```python
from build123d import *

# Parameters (mm, degrees)
BASE_BLOCK_DEPTH        = 26
UPPER_GUIDE_BLOCK_DEPTH = 30
GUIDE_SLOTS_SKETCH_W    = 26
GUIDE_SLOTS_SKETCH_H    = 5
GUIDE_SLOTS_SKETCH_W_2  = 15
GUIDE_SLOTS_SKETCH_H_2  = 20
GUIDE_SLOTS_CUT_DEPTH   = 30
OFFSET_BOSS_DEPTH       = 20
TOP_BORE_SKETCH_R       = 10
TOP_BORE_DEPTH          = 83
POCKET_SKETCH_W         = 15
POCKET_SKETCH_H         = 20
POCKET_8MM_DEEP_DEPTH   = 8
SIDE_ARCH_CUT_DEPTH     = 121
BEARING_ARCH_SKETCH_R   = 20
BEARING_ARCH_CUT_DEPTH  = 121


with BuildPart() as part:
    # Base Profile Sketch → Base Block (new body)
    with BuildSketch(Plane(origin=(0, 0, 0), x_dir=(1, 0, 0), z_dir=(0, 1, 0))):
        Polygon((50, 0), (50, 30), (-50, 30), (-50, -30), (50, -30), align=None)
    extrude(amount=BASE_BLOCK_DEPTH)

    # Upper Block Sketch → Upper Guide Block (add)
    with BuildSketch(Plane(origin=(0, 26, 0), x_dir=(1, 0, 0), z_dir=(0, 1, 0))):
        Polygon((35, 0), (35, 20), (-35, 20), (-35, -20), (35, -20), align=None)
    extrude(amount=UPPER_GUIDE_BLOCK_DEPTH)

    # Guide Slots Sketch → Guide Slots Cut (cut)
    with BuildSketch(Plane(origin=(0, 56, 0), x_dir=(1, 0, 0), z_dir=(0, 1, 0))):
        Polygon((35, 0), (35, 10), (20, 10), (20, -10), (35, -10), align=None)
        with Locations((0, -17.5)):
            Rectangle(GUIDE_SLOTS_SKETCH_W, GUIDE_SLOTS_SKETCH_H)
        with Locations((-27.5, 0)):
            Rectangle(GUIDE_SLOTS_SKETCH_W_2, GUIDE_SLOTS_SKETCH_H_2)
        with Locations((0, 17.5)):
            Rectangle(GUIDE_SLOTS_SKETCH_W, GUIDE_SLOTS_SKETCH_H)
    extrude(amount=-GUIDE_SLOTS_CUT_DEPTH, mode=Mode.SUBTRACT)

    # Offset Boss Sketch → Offset Boss (add)
    with BuildSketch(Plane.XY.offset(10)):
        Polygon((-20, 56), (-35, 26), (-20, 26), align=None)
        Polygon((20, 56), (35, 26), (20, 26), align=None)
    extrude(amount=-OFFSET_BOSS_DEPTH)

    # Top Bore Sketch → Top Bore (cut)
    with BuildSketch(Plane(origin=(0, 56, 0), x_dir=(1, 0, 0), z_dir=(0, 1, 0))):
        with Locations(Location((0, 0, 0), (0, 0, 270))):
            Circle(TOP_BORE_SKETCH_R)
    extrude(amount=-TOP_BORE_DEPTH, mode=Mode.SUBTRACT)

    # Pocket Sketch → Pocket 8mm Deep (cut)
    with BuildSketch(Plane(origin=(0, 26, 0), x_dir=(1, 0, 0), z_dir=(0, 1, 0))):
        with Locations((42.5, 0)):
            Rectangle(POCKET_SKETCH_W, POCKET_SKETCH_H)
        with Locations((-42.5, 0)):
            Rectangle(POCKET_SKETCH_W, POCKET_SKETCH_H)
    extrude(amount=-POCKET_8MM_DEEP_DEPTH, mode=Mode.SUBTRACT)

    # Side Arch Sketch → Side Arch Cut (cut)
    with BuildSketch(Plane.ZY.offset(50)):
        with BuildLine():
            Line((-15, 0), (15, 0))
            ThreePointArc((15, 0), (0, 15), (-15, 0))
        make_face()
    extrude(amount=-SIDE_ARCH_CUT_DEPTH, mode=Mode.SUBTRACT)

    # Bearing Arch Sketch → Bearing Arch Cut (cut)
    with BuildSketch(Plane(origin=(0, 0, -30), x_dir=(-1, 0, 0), z_dir=(0, 0, -1))):
        Circle(BEARING_ARCH_SKETCH_R)
    extrude(amount=-BEARING_ARCH_CUT_DEPTH, mode=Mode.SUBTRACT)


solid = part.part
```
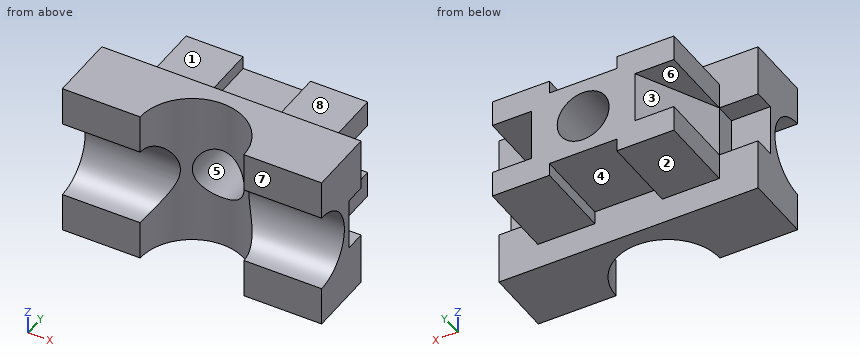
Here's how the part is built. I have some questions about the finished solid (model axes, mm). Face numbers are marked on the shaded views. A direction names the side the tool comes from. Give positions to 0.01 mm unless a question says otherwise; leave off trailing zeros. Loops run counter-clockwise (first coordinate to the right, second up) from the corner with the lowest first, then second, coordinate; pieces in that order, holes last. Notation, with made-up numbers: M -20.75,-27.75 L 7.25,-27.75 A31 cw 7.25,0.25 Z; hole C 18.5,75.5 d6. An arc over 180 degrees is marked long. Put each result on its own line as item: value. Start each with the question number.
(1) I want a section at C-C on x = 0. Please give me the cut outline in (y, z).
(2) I need wall thicknesses on line 1 along X through (y, z) = (36, 0); line 2 along X through (y, z) = (38, 17); line 3 along Z through (x, y) = (0, 27.5). Which ranges of each line are inside material? Lowest first, please. Write a range as [from, to].
(3) If we mould it in two halves opening along Z, with no side actions, what happens to the marked faces 5, 6, 7 and 8? For each: +Z half, -Z half, draft (parallel to the pull), parting line (faces both ways), or undercut.
(4) I want a section at D-D on x = 33. Please give me the cut outline in (y, z).
(5) I want a section at B-B on y = 48. Please give me the cut outline in (x, z).
(6) For the marked faces 1, 2, 3 and 4, which set-ups out of +Z, -Z, +X, -X, +Y, -Y let a thin tool reach every point of the face, with its end or its side?
(7) Will these pins go through, and if not, where does the flat tip stop? pin 1 Ø4 at (y, z) = (40.5, 17) entering from -X; pin 2 Ø11 at (y, z) = (38, -16.5) entering from +X; pin 3 Ø3 at (x, z) = (3.5, 19) entering from +Y; pin 4 Ø8 at (y, z) = (21, -7) entering from +X.
(8) I want a section at A-A on z = 0. Please give me the cut outline in (x, y).
Answer block:
1. outline: M 20,-30 L 26,-30 L 26,-15 L 56,-15 L 56,-10 L 20,-10 Z; M 20,10 L 56,10 L 56,15 L 26,15 L 26,30 L 20,30 Z
2. line 1: [-30, -10], [10, 30]
2. line 2: [-35, -13], [13, 35]
2. line 3: [-15, -10], [10, 15]
3. face 5: undercut
3. face 6: undercut
3. face 7: draft
3. face 8: +Z half
4. outline: M 0,-30 L 26,-30 L 26,-20 L 56,-20 L 56,-10 L 30,-10 L 30,10 L 56,10 L 56,20 L 26,20 L 26,30 L 0,30 L 0,15 A15 cw 0,-15 Z
5. outline: M -35,-20 L -13,-20 L -13,-15 L 13,-15 L 13,-20 L 35,-20 L 35,-10 L 24,-10 L 24,10 L 35,10 L 35,20 L 13,20 L 13,15 L -13,15 L -13,20 L -35,20 L -35,10 L -24,10 L -24,-10 L -35,-10 Z; hole C 0,0 d20
6. face 1: +Z, +X, -X, +Y
6. face 2: -Z, +X, -X, +Y
6. face 3: -X, +Y
6. face 4: -Z, +Y
7. pin 1: x = -35
7. pin 2: x = 35
7. pin 3: y = 26
7. pin 4: x = 50
8. outline: M -50,15 L -13.23,15 A20 cw -10,17.32 L -10,56 L -20,56 L -35,26 L -35,18 L -50,18 Z; M 10,17.32 A20 cw 13.23,15 L 50,15 L 50,18 L 35,18 L 35,26 L 20,56 L 10,56 Z
